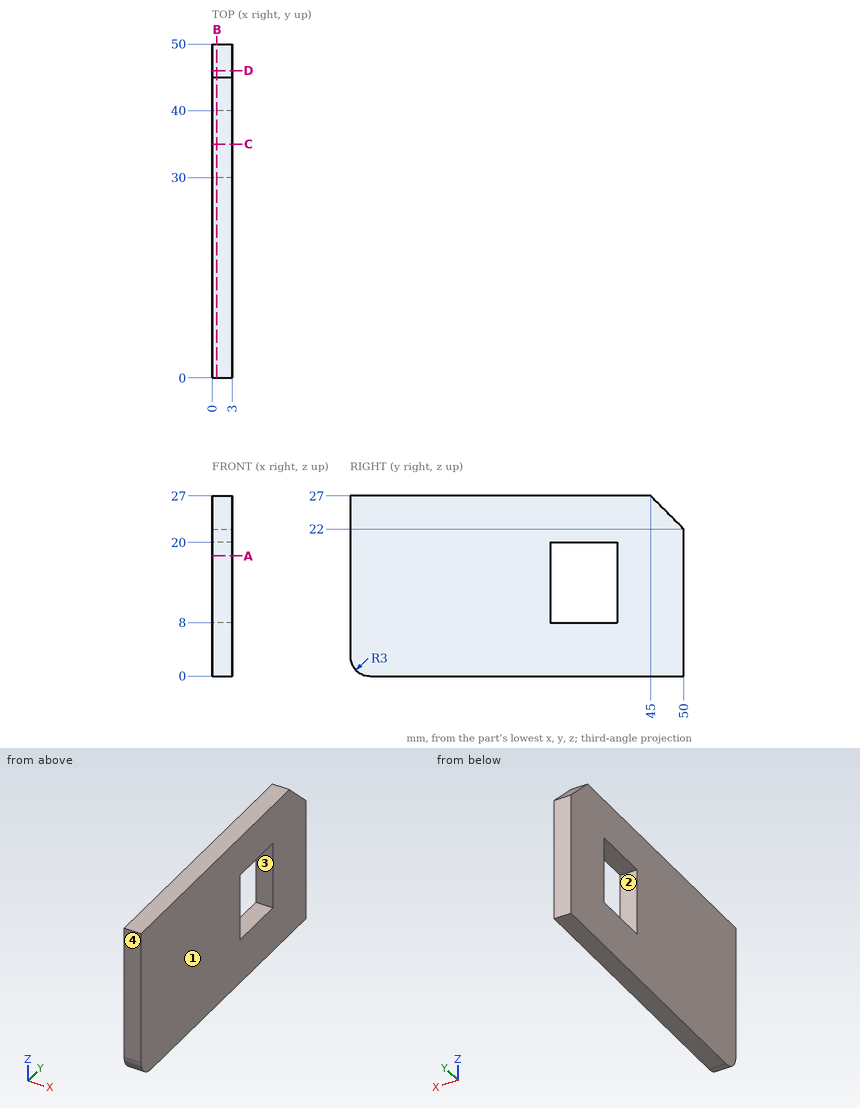
Here's the drawing with two shaded views (mm, measured from the low corner). I have some questions. Give positions to 0.01 mm unless a question says otherwise; leave off trailing zeros. Loops run counter-clockwise (first coordinate to the right, second up) from the corner with the lowest first, then second, coordinate; pieces in that order, holes last. Notation, with made-up numbers: M -4,47.5 L 51,47.5 A25 cw 51,82.5 Z; hole C 67.5,22 d11. An arc over 180 degrees is marked long. One line per item, written item: value. Start each with the question number.
1) If we section it at A-A, the plane z = 18: Write out the boundary of the cut face in (x, y).
2) If we section it at C-C, the plane y = 35: Write out the boundary of the cut face in (x, z).
3) If we section it at D-D, the plane y = 46: Write out the boundary of the cut face in (x, z), and give its area (3 significant figures).
4) I'm going to push a flat-ended pin straight in: pin 1 (5 mm diameter, centred on y = 5.5, z = 11.5, fed in from -X). Where does the tip first touch, or does it pass through?
5) If I drill on line 1 (Z direction, x = 2.1, y = 36.5); line 2 (Y direction, x = 1.25, z = 13.25); line 3 (Y direction, x = 0.2, z = 25.5), over which ranges is the centre line in solid material (lowest first)? Write a range as [from, to].
6) Thinking about a two-plate mould opening in Y: for the marked faces 1, 2, 3 and 4, which applies, +Y half, -Y half, draft (parallel to the pull), parting line (faces both ways), or undercut?
7) If we section it at B-B, the plane x = 0.7: Write out the boundary of the cut face in (y, z), and give its area (3 significant figures).
Completed:
1. outline: M 0,0 L 3,0 L 3,30 L 0,30 Z; M 0,40 L 3,40 L 3,50 L 0,50 Z
2. outline: M 0,0 L 3,0 L 3,8 L 0,8 Z; M 0,20 L 3,20 L 3,27 L 0,27 Z
3. outline: M 0,0 L 3,0 L 3,26 L 0,26 Z
3. area: 78.0 mm^2
4. pin 1: stops at x = 0
5. line 1: z = [0, 8], [20, 27]
5. line 2: y = [0, 30], [40, 50]
5. line 3: y = [0, 46.5]
6. face 1: draft
6. face 2: undercut
6. face 3: undercut
6. face 4: -Y half
7. outline: M 0,3 A3 ccw 3,0 L 50,0 L 50,22 L 45,27 L 0,27 Z; hole M 30,8 L 40,8 L 40,20 L 30,20 Z
7. area: 1,220 mm^2
